Verification items for the finished model (mm, model axes). Face numbers are marked on the shaded views. A direction names the side the tool comes from. Give positions to 0.01 mm unless a question says otherwise; leave off trailing zeros. Loops run counter-clockwise (first coordinate to the right, second up) from the corner with the lowest first, then second, coordinate; pieces in that order, holes last. Notation, with made-up numbers: M 13,42 L 23,42 A22 cw 23,79 Z; hole C 71.25,39.25 d10. An arc over 180 degrees is marked long. Use a Markdown table: item, result.
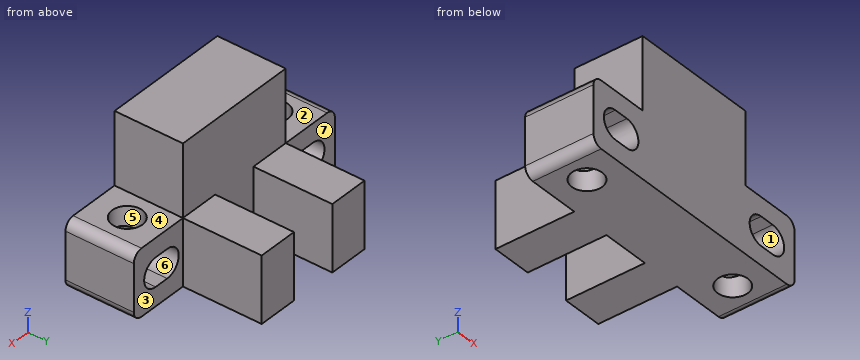
from build123d import *

# Parameters (mm, degrees)
EXTRUDE_1_DEPTH     = 7.2
SKETCH_2_W          = 4.2
SKETCH_2_H          = 6.94
EXTRUDE_2_DEPTH     = 8.3
CUT_EXTRUDE_1_DEPTH = 32.073783162
SKETCH_4_R          = 1.6
CUT_EXTRUDE_2_DEPTH = 32.366281259
FILLET_1_R          = 1


with BuildPart() as part:
    # 草图1 → 凸台-拉伸1 (new body)
    with BuildSketch(Plane(origin=(0, 0, 0), x_dir=(1, 0, 0), z_dir=(0, 1, 0))):
        Polygon((0, -6.94), (6.4, -6.94), (6.4, -14.5), (19.8, -14.5), (19.8, -6.94), (26.2, -6.94), (26.2, 0), (0, 0), align=None)
    extrude(amount=EXTRUDE_1_DEPTH)

    # 草图2 → 凸台-拉伸2 (add)
    with BuildSketch(Plane(origin=(0, 7.2, 0), x_dir=(1, 0, 0), z_dir=(0, 1, 0))):
        with Locations((8.5, -3.47)):
            Rectangle(SKETCH_2_W, SKETCH_2_H)
        with Locations((17.7, -3.47)):
            Rectangle(SKETCH_2_W, SKETCH_2_H)
    extrude(amount=EXTRUDE_2_DEPTH)

    # 草图3 → 切除-拉伸1 (cut, through all)
    with BuildSketch(Plane(origin=(0, 7.2, 0), x_dir=(1, 0, 0), z_dir=(0, 1, 0))):
        with BuildLine():
            Line((2.85, -1.97), (4.35, -1.97))
            ThreePointArc((4.35, -1.97), (5.85, -3.47), (4.35, -4.97))
            Line((4.35, -4.97), (2.85, -4.97))
            ThreePointArc((2.85, -4.97), (1.35, -3.47), (2.85, -1.97))
        make_face()
        with BuildLine():
            Line((23.35, -4.97), (21.85, -4.97))
            ThreePointArc((21.85, -4.97), (20.35, -3.47), (21.85, -1.97))
            Line((21.85, -1.97), (23.35, -1.97))
            ThreePointArc((23.35, -1.97), (24.85, -3.47), (23.35, -4.97))
        make_face()
    extrude(amount=-CUT_EXTRUDE_1_DEPTH, mode=Mode.SUBTRACT)

    # 草图4 → 切除-拉伸2 (cut, through all)
    with BuildSketch(Plane.XY.offset(6.94)):
        with Locations((22.6, 3.6)):
            Circle(SKETCH_4_R)
        with Locations((3.6, 3.6)):
            Circle(SKETCH_4_R)
    extrude(amount=-CUT_EXTRUDE_2_DEPTH, mode=Mode.SUBTRACT)

    # 圆角1
    fillet_1_edges = [part.edges().sort_by_distance(p)[0] for p in [
        (0, 3.6, 0),
        (0, 3.6, 6.94),
        (26.2, 3.6, 0),
        (26.2, 3.6, 6.94),
    ]]
    fillet(fillet_1_edges, radius=FILLET_1_R)


solid = part.part
(1) Set-up check for the marked faces 1, 2, 3 and 4: record each of +Z, -Z, +X, -X, +Y, -Y from which the full face is reachable in a straight line by a thin tool's end or side.
Results below:
| item | result |
|---|---|
| face 1 | +Y, -Y |
| face 2 | +Z, -X, +Y, -Y |
| face 3 | +Z, -Z, +X, +Y |
| face 4 | +Z, +X, +Y, -Y |
(2) Cross-section at A-A on y = 12.5. Record the cut outline in (x, z), then the cut area to 3 significant figures.
Results below:
| item | result |
|---|---|
| outline | M 6.4,0 L 10.6,0 L 10.6,6.94 L 6.4,6.94 Z; M 15.6,0 L 19.8,0 L 19.8,6.94 L 15.6,6.94 Z |
| area | 58.3 mm^2 |
(3) Cross-section at B-B on y = 1.5. Record the cut outline in (x, z), then the cut area to 3 significant figures.
Results below:
| item | result |
|---|---|
| outline | M 0,1 A1 ccw 1,0 L 25.2,0 A1 ccw 26.2,1 L 26.2,5.94 A1 ccw 25.2,6.94 L 19.8,6.94 L 19.8,14.5 L 6.4,14.5 L 6.4,6.94 L 1,6.94 A1 ccw 0,5.94 Z; hole M 2.85,1.97 L 4.35,1.97 A1.5 ccw 4.35,4.97 L 2.85,4.97 A1.5 ccw Z; hole M 21.85,1.97 L 23.35,1.97 A1.5 ccw 23.35,4.97 L 21.85,4.97 A1.5 ccw Z |
| area | 259 mm^2 |
(4) Material ranges on line 1 (X direction, y = 12.5, z = 5); line 2 (Y direction, x = 22.6, z = 1.45); line 3 (X direction, y = 3.6, z = 5.9), recorded low to high.
Results below:
| item | result |
|---|---|
| line 1 | 6.4 to 10.6, 15.6 to 19.8 |
| line 2 | 0 to 2, 5.2 to 7.2 |
| line 3 | 0 to 2, 5.2 to 21, 24.2 to 26.2 |
(5) Draft check along Y on the marked faces 5, 6 and 7. Enter one of: +Y half, -Y half, draft (parallel to the pull), parting line (faces both ways), or undercut.
Results below:
| item | result |
|---|---|
| face 5 | undercut |
| face 6 | draft |
| face 7 | +Y half |
(6) Cross-section at D-D on y = 3.6. Record the cut outline in (x, z).
Results below:
| item | result |
|---|---|
| outline | M 0,1 A1 ccw 1,0 L 2,0 L 2,2.23 A1.5 cw 2,4.71 L 2,6.94 L 1,6.94 A1 ccw 0,5.94 Z; M 5.2,0 L 21,0 L 21,2.23 A1.5 cw 21,4.71 L 21,6.94 L 19.8,6.94 L 19.8,14.5 L 6.4,14.5 L 6.4,6.94 L 5.2,6.94 L 5.2,4.71 A1.5 cw 5.2,2.23 Z; M 24.2,0 L 25.2,0 A1 ccw 26.2,1 L 26.2,5.94 A1 ccw 25.2,6.94 L 24.2,6.94 L 24.2,4.71 A1.5 cw 24.2,2.23 Z |
(7) Gauge pin test, flat ends, axial feed: P1, Ø1.9, axis at x = 22.5, z = 4.5, coming from the +Y side; P2, Ø4, axis at y = 4.5, z = 10, coming from the -X side; P3, Ø5.5, axis at y = 12.5, z = 5, coming from the +X side. Record the tip position at first contact, or that the pin passes through.
Results below:
| item | result |
|---|---|
| P1 | y = 7.2 |
| P2 | x = 6.4 |
| P3 | x = 19.8 |
(8) Cross-section at C-C on z = 5.5. Record the cut outline in (x, y).
Results below:
| item | result |
|---|---|
| outline | M 0,0 L 26.2,0 L 26.2,7.2 L 19.8,7.2 L 19.8,15.5 L 15.6,15.5 L 15.6,7.2 L 10.6,7.2 L 10.6,15.5 L 6.4,15.5 L 6.4,7.2 L 0,7.2 Z; hole C 3.6,3.6 d3.2; hole C 22.6,3.6 d3.2 |
